For this review, take the finished solid that the model builds, in its own axes (mm). A direction names the side the tool comes from. Coordinates: 2 decimals unless noted, no trailing zeros. Write each loop counter-clockwise with the first axis right and the second up, starting at its lowest first coordinate (ties: lowest second). Pieces come first, ordered by that corner, then holes. Notation, with made-up numbers: (-13, 59) -> (4, 59) arc R26 ccw to (4, 92) -> close; hole circle Ø1 at (-20.5, 41.25). An arc over 180 degrees is marked (long way). One line per item, written item: value. Start each with the question number.
1) Add section A-A (x = 252). State the section outline as (y, z) points.
2) Machinability: for faces 1 (the flat face through (412.5, -7, -20)), 2 (the flat face through (402.5, -7, -25)), 3 (the flat face through (-240, 0, 1)), 4 (the flat face through (-6, -8, 10)), 5 (the flat face through (242, 0, 3)), which of the approach directions +Z, -Z, +X, -X, +Y, -Y give a long, thin tool a straight path to every point of the face, cutting with its end or side? Answer none if there is none.
3) Mouldability with a two-part tool opening along X and no side actions: class faces 6 (the flat face through (-402.5, -7, -25)), 7 (the flat face through (-412.5, -7, -20)), 8 (the flat face through (2, -15, 5)), 9 (the flat face through (-6, -8, 0)) as released by +X, released by -X, zero draft, split by the parting line, or undercut.
4) For probe 1 along Y at (x, z) = (-407, -35); probe 2 along X at (y, z) = (-5.5, -25.5); probe 3 along Y at (x, z) = (0, 6), list the stretches that pass through material, from the lowest coordinate up. Write a range as from..to.
5) For pin 1 Ø8 at (x, z) = (176.5, -7.5) entering from -Y; pin 2 Ø7.5 at (x, y) = (174.5, 0) entering from -Z; pin 3 Ø16.5 at (x, z) = (277.5, -4) entering from +Y, all flat-tipped, find the tip position at first contact; note any pin that passes through.
from build123d import *

# Parameters (mm, degrees)
SKETCH_1_R      = 5
EXTRUDE_1_DEPTH = 10
SKETCH_2_W      = 45
SKETCH_2_H      = 15
SKETCH_2_R      = 4
EXTRUDE_2_DEPTH = 10
EXTRUDE_START   = -10
SKETCH_3_W      = 45
SKETCH_3_H      = 15
SKETCH_3_R      = 4
EXTRUDE_3_DEPTH = 10
FILLET_1_R      = 5


with BuildPart() as part:
    # 草图1 → 凸台-拉伸1 (new body)
    with BuildSketch(Plane.XY):
        with BuildLine():
            Line((0, -15), (412.5, -15))
            Line((412.5, -15), (412.5, 0))
            Line((412.5, 0), (10, 0))
            ThreePointArc((10, 0), (0, 10), (-10, 0))
            Line((-10, 0), (-412.5, 0))
            Line((-412.5, 0), (-412.5, -15))
            Line((-412.5, -15), (0, -15))
        make_face()
        Circle(SKETCH_1_R, mode=Mode.SUBTRACT)
    extrude(amount=EXTRUDE_1_DEPTH)

    # 草图2 → 凸台-拉伸2 (add)
    with BuildSketch(Plane(origin=(412.5, 0, 0), x_dir=(0, 0, -1), z_dir=(1, 0, 0))):
        with Locations((22.5, -7.5)):
            Rectangle(SKETCH_2_W, SKETCH_2_H)
        with Locations((15, -7.5)):
            Circle(SKETCH_2_R, mode=Mode.SUBTRACT)
        with Locations((35, -7.5)):
            Circle(SKETCH_2_R, mode=Mode.SUBTRACT)
    extrude(amount=-EXTRUDE_2_DEPTH)

    # 草图3 → 凸台-拉伸3 (add)
    with BuildSketch(Plane.ZY.offset(412.5).offset(EXTRUDE_START)):
        with Locations((-22.5, -7.5)):
            Rectangle(SKETCH_3_W, SKETCH_3_H)
        with Locations(Location((-35, -7.5, 0), (0, 0, 180))):
            Circle(SKETCH_3_R, mode=Mode.SUBTRACT)
        with Locations(Location((-15, -7.5, 0), (0, 0, 180))):
            Circle(SKETCH_3_R, mode=Mode.SUBTRACT)
    extrude(amount=EXTRUDE_3_DEPTH)

    # 圆角1
    fillet_1_edges = [part.edges().sort_by_distance(p)[0] for p in [
        (-412.5, -7.5, 10),
        (402.5, -7.5, 0),
        (412.5, -7.5, 10),
        (-402.5, -7.5, 0),
    ]]
    fillet(fillet_1_edges, radius=FILLET_1_R)


solid = part.part
Numbers:
1. outline: (-15, 0) -> (0, 0) -> (0, 10) -> (-15, 10) -> close
2. face 1: +Z, -Z, +X, +Y, -Y
2. face 2: -Z, +Y, -Y
2. face 3: +Z, -Z, -X, +Y
2. face 4: +Z, +X, -X, +Y, -Y
2. face 5: +Z, -Z, +X, +Y
3. face 6: undercut
3. face 7: released by -X
3. face 8: zero draft
3. face 9: undercut
4. probe 1: -15..-11.5, -3.5..0
4. probe 2: -412.5..-402.5, 402.5..412.5
4. probe 3: -15..-5, 5..10
5. pin 1: through
5. pin 2: z = 0
5. pin 3: y = 0
